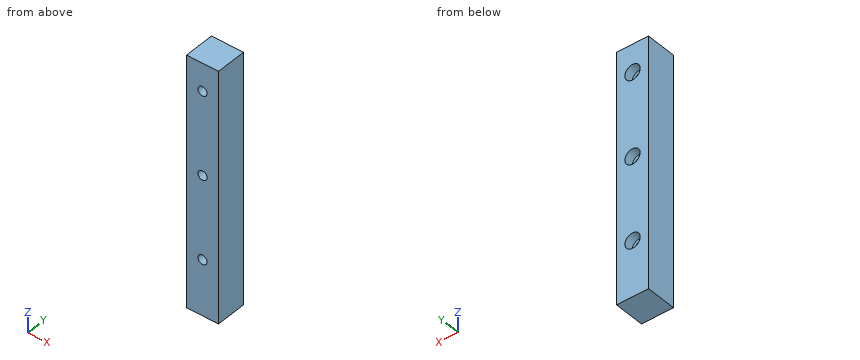
```python
from build123d import *

# Parameters (mm, degrees)
SKETCH_1_W                   = 23
SKETCH_1_H                   = 22
EXTRUDE_1_DEPTH              = 180
HOLE_WIZARD_M6_1_D           = 6.6
HOLE_WIZARD_M6_1_CBORE_D     = 11
HOLE_WIZARD_M6_1_CBORE_DEPTH = 6.4
PATTERN_LINEAR_1_COUNT       = 4
PATTERN_LINEAR_1_PITCH       = 60


with BuildPart() as part:
    # 草图1 → 凸台-拉伸1 (new body)
    with BuildSketch(Plane.XY):
        with Locations((11.5, 11)):
            Rectangle(SKETCH_1_W, SKETCH_1_H)
    extrude(amount=EXTRUDE_1_DEPTH)

    # M6 六角凹头螺钉的柱形沉头孔1 (through all)
    with Locations(Plane(origin=(0, 22, 0), x_dir=(1, 0, 0), z_dir=(0, 1, 0))):
        with Locations((11.5, -160)):
            hole_wizard_m6_1 = CounterBoreHole(HOLE_WIZARD_M6_1_D / 2, HOLE_WIZARD_M6_1_CBORE_D / 2, HOLE_WIZARD_M6_1_CBORE_DEPTH)

    # 阵列(线性)1: M6 六角凹头螺钉的柱形沉头孔1 ×4
    with Locations(*[(0, 0, -i * PATTERN_LINEAR_1_PITCH) for i in range(1, PATTERN_LINEAR_1_COUNT)]):
        add(hole_wizard_m6_1, mode=Mode.SUBTRACT)


solid = part.part
```
Input: part model. Units: mm. Frame: model coordinates. Give positions to 0.01 mm unless a question says otherwise; leave off trailing zeros. Order: outer loops, then holes, each group sorted by start corner. A loop starts at its lowest first (then second) coordinate and runs counter-clockwise, first axis right, second up. Notation, with made-up numbers: (78, 67) - (109, 67) arc R30 cw to (109, 90) - close; hole circle Ø4 at (-32, 20). An arc over 180 degrees is marked (long way). Put each result on its own line as item: value.
Item 1: Section query B-B, the plane y = 8.5. Return loops of the section in (x, z).
Found:
outline: (0, 0) - (23, 0) - (23, 180) - (0, 180) - close; hole circle Ø6.6 at (11.5, 40); hole circle Ø6.6 at (11.5, 100); hole circle Ø6.6 at (11.5, 160)
Item 2: Section query A-A, the plane z = 100. Return loops of the section in (x, y), then the cut area to 3 significant figures.
Found:
outline: (0, 0) - (8.2, 0) - (8.2, 15.6) - (6, 15.6) - (6, 22) - (0, 22) - close; (14.8, 0) - (23, 0) - (23, 22) - (17, 22) - (17, 15.6) - (14.8, 15.6) - close
area: 333 mm^2
Item 3: Contact query for flat-ended pins moving along their axis: pin 1 (4 mm diameter, centred on x = 11.5, z = 160, fed in from +Y); pin 2 (10 mm diameter, centred on x = 11.5, z = 100, fed in from +Y). Output: stop coordinate, or through.
Found:
pin 1: passes through
pin 2: stops at y = 15.6
Item 4: Ray query, L1, parallel to Z at x = 11.5, y = 20; L2, parallel to Z at x = 11.5, y = 12.5; L3, parallel to X at y = 20.5, z = 100. Return the intervals inside material, ascending. Write a range as from..to.
Found:
L1: z = 0..34.5, 45.5..94.5, 105.5..154.5, 165.5..180
L2: z = 0..36.7, 43.3..96.7, 103.3..156.7, 163.3..180
L3: x = 0..6, 17..23
Item 5: Section query C-C, the plane x = 11.5. Return loops of the section in (y, z), then the cut area to 3 significant figures.
Found:
outline: (0, 0) - (22, 0) - (22, 34.5) - (15.6, 34.5) - (15.6, 36.7) - (0, 36.7) - close; (0, 43.3) - (15.6, 43.3) - (15.6, 45.5) - (22, 45.5) - (22, 94.5) - (15.6, 94.5) - (15.6, 96.7) - (0, 96.7) - close; (0, 103.3) - (15.6, 103.3) - (15.6, 105.5) - (22, 105.5) - (22, 154.5) - (15.6, 154.5) - (15.6, 156.7) - (0, 156.7) - close; (0, 163.3) - (15.6, 163.3) - (15.6, 165.5) - (22, 165.5) - (22, 180) - (0, 180) - close
area: 3,440 mm^2
